Read the model definition and answer for the solid it produces. Units are mm, in the model's axes. A direction names the side the tool comes from. Coordinates: 2 decimals unless noted, no trailing zeros. Loops run counter-clockwise (first coordinate to the right, second up) from the corner with the lowest first, then second, coordinate; pieces in that order, holes last. Notation, with made-up numbers: (47.5, 61) -> (94.5, 61) arc R9 ccw to (94.5, 76) -> close; hole circle Ø3 at (34.25, 83). An arc over 180 degrees is marked (long way). Answer as CSV lines item,"result".
```python
from build123d import *

# Parameters (mm, degrees)
G1_2_TAPPED_HOLE1_D                               = 19
HOLE_SIZE_BASED_ON_SOCKET_HEAD_CAP_SC_D           = 4.8
HOLE_SIZE_BASED_ON_SOCKET_HEAD_CAP_SC_CBORE_D     = 8
HOLE_SIZE_BASED_ON_SOCKET_HEAD_CAP_SC_CBORE_DEPTH = 4.6
CHAMFER1_SIZE                                     = 0.2
CHAMFER2_SIZE                                     = 0.2
SKETCH7_OUTSIDE_W                                 = 67.362
SKETCH7_OUTSIDE_H                                 = 67.362
CUT_EXTRUDE1_DEPTH                                = 50


with BuildPart() as part:
    # Sketch2 → Revolve1 (revolve)
    with BuildSketch(Plane.XY, mode=Mode.PRIVATE) as revolve1_sk:
        Polygon((0, 30), (-25, 30), (-25, 22), (-14.25, 22), (-14.25, 0), (0, 0), align=None)
    revolve(revolve1_sk.sketch.rotate(Axis((0, 0, 0), (0, 1, 0)), 270), axis=Axis((0, 0, 0), (0, 1, 0)))

    # G1/2 Tapped Hole1 (through all)
    with Locations(Plane.ZX.offset(30)):
        with Locations((0, 0)):
            Hole(G1_2_TAPPED_HOLE1_D / 2)

    # Hole Size (% based on) Socket Head Cap Screw Type 1 (through all)
    with Locations(Plane(origin=(-12.727922061, 30, -12.727922061), x_dir=(0, 0, 1), z_dir=(0, 1, 0))):
        with Locations((0, 0), (25.455844122, 25.455844122)):
            CounterBoreHole(HOLE_SIZE_BASED_ON_SOCKET_HEAD_CAP_SC_D / 2, HOLE_SIZE_BASED_ON_SOCKET_HEAD_CAP_SC_CBORE_D / 2, HOLE_SIZE_BASED_ON_SOCKET_HEAD_CAP_SC_CBORE_DEPTH)

    # Chamfer1
    chamfer1_edges = [part.edges().sort_by_distance(p)[0] for p in [
        (0, 0, 14.25),
        (0, 22, 25),
        (0, 30, 25),
    ]]
    chamfer(chamfer1_edges, length=CHAMFER1_SIZE)

    # Chamfer2
    chamfer2_edges = [part.edges().sort_by_distance(p)[0] for p in [
        (0, 22, 14.25),
    ]]
    chamfer(chamfer2_edges, length=CHAMFER2_SIZE)

    # Sketch7 outside → Cut-Extrude1 (cut)
    with BuildSketch(Plane(origin=(0, 30, 0), x_dir=(1, 0, 0), z_dir=(0, 1, 0))):
        Rectangle(SKETCH7_OUTSIDE_W, SKETCH7_OUTSIDE_H)
        Polygon((-24.748737342, 45.961940777), (45.961940777, -24.748737342), (24.748737342, -45.961940777), (-45.961940777, 24.748737342), align=None, mode=Mode.SUBTRACT)
    extrude(amount=-CUT_EXTRUDE1_DEPTH, mode=Mode.SUBTRACT)


solid = part.part
```
Q1. A cutting plane is placed at C-C, the plane y = 9.25. Write down the section's boundary in (x, z).
Results:
outline,"circle Ø28.5 at (0, 0); hole circle Ø19 at (0, 0)"
Q2. For faces 5 (the face through (12.8, 25.4, 15.3)), 6 (the face through (-8.43, 14.79, -4.38)), determine the directions among +Z, -Z, +X, -X, +Y, -Y from which every point of the face is accessible in a straight line to the end or side of a thin tool.
Results:
face 5,"+Y"
face 6,"+Y, -Y"
Q3. Find the intervals of material crossed by probe 1 along X at (y, z) = (9.5, 0.5); probe 2 along X at (y, z) = (11.25, 8.5); probe 3 along Z at (x, y) = (3.5, 16.75), in increasing order. Write a range as [from, to].
Results:
probe 1,"x = [-14.24, -9.49], [9.49, 14.24]"
probe 2,"x = [-11.44, -4.24], [4.24, 11.44]"
probe 3,"z = [-13.81, -8.83], [8.83, 13.81]"
Q4. A cutting plane is placed at B-B, the plane z = 0. Write down the section's boundary in (x, y), and give its area (3 significant figures).
Results:
outline,"(-21.21, 22) -> (-14.45, 22) -> (-14.25, 21.8) -> (-14.25, 0.2) -> (-14.05, 0) -> (-9.5, 0) -> (-9.5, 30) -> (-21.21, 30) -> close; (9.5, 0) -> (14.05, 0) -> (14.25, 0.2) -> (14.25, 21.8) -> (14.45, 22) -> (21.21, 22) -> (21.21, 30) -> (9.5, 30) -> close"
area,"396 mm²"
Q5. A cutting plane is placed at A-A, the plane x = 0. Write down the section's boundary in (y, z).
Results:
outline,"(0, -14.05) -> (0.2, -14.25) -> (21.8, -14.25) -> (22, -14.45) -> (22, -21.21) -> (30, -21.21) -> (30, -9.5) -> (0, -9.5) -> close; (0, 9.5) -> (30, 9.5) -> (30, 21.21) -> (22, 21.21) -> (22, 14.45) -> (21.8, 14.25) -> (0.2, 14.25) -> (0, 14.05) -> close"
Q6. For a pull along Z with two mould halves and no side action, classify faces 1 (the face through (13.91, 10.85, 3.09)), 2 (the face through (-17.518, 25.947, -17.836)), 3 (the face through (11.81, 23.68, 10.51)), 4 (the face through (-16.277, 27.732, -10.882)) as pulls with the +Z half, pulls with the -Z half, needs draft (parallel to the pull), parting line crosses it, or undercut.
Results:
face 1,"parting line crosses it"
face 2,"pulls with the -Z half"
face 3,"undercut"
face 4,"undercut"
Q7. Given pin 1 Ø5.5 at (x, z) = (12.73, 12.73) entering from -Y; pin 2 Ø4 at (y, z) = (19.5, 0.5) entering from -X; pin 3 Ø8 at (y, z) = (4, 15) entering from +X; pin 4 Ø2 at (y, z) = (3.5, 17) entering from -X, each flat-ended and moving along its own axis, determine where each tip first touches the part or whether it passes through.
Results:
pin 1,"stops at y = 22"
pin 2,"stops at x = -14.25"
pin 3,"stops at x = 9.06"
pin 4,"passes through"
